from build123d import *


with BuildPart() as part:
    # Sketch1 → Revolve1 (revolve)
    with BuildSketch(Plane(origin=(0, 0, 0), x_dir=(1, 0, 0), z_dir=(0, 1, 0)), mode=Mode.PRIVATE) as revolve1_sk:
        with BuildLine():
            Line((-15.545938878, 0), (-15.545938878, 6))
            Line((-15.545938878, 6), (-15.045938878, 6.5))
            Line((-15.045938878, 6.5), (-6.045938878, 6.5))
            Line((-6.045938878, 6.5), (-5.545938878, 6))
            Line((-5.545938878, 6), (-5.545938878, 3))
            Line((-5.545938878, 3), (-2.680089485, 3))
            Line((-2.680089485, 3), (-2.680089485, 5))
            Line((-2.680089485, 5), (-1.680089485, 6))
            Line((-1.680089485, 6), (-0.680089485, 6))
            Line((-0.680089485, 6), (-0.680089485, 4.5))
            Line((-0.680089485, 4.5), (0.319910515, 4.5))
            Line((0.319910515, 4.5), (0.319910515, 4.75))
            Line((0.319910515, 4.75), (9.319910515, 4.75))
            Line((9.319910515, 4.75), (9.319910515, 3))
            Line((9.319910515, 3), (13.954061122, 3))
            Line((13.954061122, 3), (14.454061122, 2.5))
            Line((14.454061122, 2.5), (14.454061122, 2))
            ThreePointArc((14.454061122, 2), (15.868274684, 1.414213562), (16.454061122, 0))
            Line((16.454061122, 0), (-15.545938878, 0))
        make_face()
    revolve(revolve1_sk.sketch.rotate(Axis((-122.432679922, 0, 0), (1, 0, 0)), 180), axis=Axis((-122.432679922, 0, 0), (1, 0, 0)))


solid = part.part
The listing builds one solid part. Answer for the finished solid, in the listing's coordinates (mm). A direction names the side the tool comes from. Give positions to 0.01 mm unless a question says otherwise; leave off trailing zeros. Write each loop counter-clockwise with the first axis right and the second up, starting at its lowest first coordinate (ties: lowest second). Pieces come first, ordered by that corner, then holes.
Item 1: Section C-C, the plane x = -10.5 is taken. Write down the section's boundary in (y, z), plus the area to 3 significant figures.
Item 2: Determine the mould class of faces 1 (the cylindrical face through (-0.17, -3.04, -3.32)), 2 (the cylindrical face through (4.883, 4.637, -1.03)), 3 (the flat face through (-15.546, 0, 0)), 4 (the flat face through (14.454, -2, -1)) for opening direction X: released by +X, released by -X, zero draft, split by the parting line, or undercut.
Item 3: Section D-D, the plane x = 7 is taken. Write down the section's boundary in (y, z), plus the area to 3 significant figures.
Item 4: Find the intervals of material crossed by line 1 along X through (y, z) = (2.75, 1.75); line 2 along X through (y, z) = (2, -0.75); line 3 along X through (y, z) = (-2.75, 4.75), in increasing order.
Item 5: Flat-ended cylindrical pins translate along their axes: P1, Ø1.5, axis at y = -1, z = -0.5, coming from the +X side; P2, Ø3, axis at y = 2.5, z = -1, coming from the +X side; P3, Ø1, axis at x = -1, y = 4.5, coming from the +Z side. Find the tip coordinate at first contact, or state that the pin passes through.
Item 6: Which of the six approach directions +Z, -Z, +X, -X, +Y, -Y give full straight-line access (tool end or side, diameter ignored) to faces 5 (the cylindrical face through (-10.483, 3.955, -5.158)), 6 (the cylindrical face through (-1.173, -1.802, 5.723)), 7 (the cylindrical face through (-4.09, -0.9, 2.86))?
Completed:
1. outline: circle Ø13 at (0, 0)
1. area: 133 mm2
2. face 1: undercut
2. face 2: zero draft
2. face 3: released by -X
2. face 4: released by +X
3. outline: circle Ø9.5 at (0, 0)
3. area: 70.9 mm2
4. line 1: x = -15.55 to -5.55, -2.68 to 9.32
4. line 2: x = -15.55 to 14.45
4. line 3: x = -15.55 to -5.55, -2.19 to -0.68
5. P1: stops at x = 16.42
5. P2: stops at x = 16.06
5. P3: stops at z = 4.47
6. face 5: +X, -X
6. face 6: +X
6. face 7: none
